Design review of the part built by this model. Coordinates are the model's own, in mm. A direction names the side the tool comes from. Give positions to 0.01 mm unless a question says otherwise; leave off trailing zeros. Write each loop counter-clockwise with the first axis right and the second up, starting at its lowest first coordinate (ties: lowest second). Pieces come first, ordered by that corner, then holes. Notation, with made-up numbers: (84.25, -36.75) -> (110.25, -36.75) arc R13 ccw to (110.25, -17.75) -> close; hole circle Ø4 at (57.25, 76). An arc over 180 degrees is marked (long way). Write each question's results on one line, items separated by ' | '. Start each with the question number.
(1) To check wall thickness, follow probe 1 along Z at (x, y) = (-37.5, 3.25); probe 2 along Z at (x, y) = (-12.5, 16.25); probe 3 along X at (y, z) = (10.25, 7). State the ranges of each line that lie inside material, in increasing order.
(2) Mouldability with a two-part tool opening along Z and no side actions: class faces 4 (the face through (-49.156, 16.181, 49.527)), 5 (the face through (-38.13, 12.98, 38.33)), 6 (the face through (62.5, 5, 0)) as released by +Z, released by -Z, zero draft, split by the parting line, or undercut.
(3) For faces 1 (the face through (-41.15, 5.07, 32.74)), 2 (the face through (53.479, 5.07, 53.945)), 3 (the face through (-7.441, 14.93, 9.274)), list the 3-axis set-ups (+Z, -Z, +X, -X, +Y, -Y) from which the entire face can be reached by the end or side of a thin tool; tool diameter is ignored.
(4) Take a section at A-A (y = 4.5). State the section outline as (x, z) points, plus the area to 3 significant figures.
(5) Take a section at B-B (x = -21.5). State the section outline as (y, z) points.
(6) Take a section at C-C (z = 27.5). State the section outline as (x, y) points.
(7) Clearance check with flat-ended pins moving along their axes: pin 1 (6 mm diameter, centred on x = -41, y = 2.5, fed in from +Z); pin 2 (12 mm diameter, centred on x = 47.5, y = 14.5, fed in from -Z); pin 3 (3 mm diameter, centred on y = 14, z = 6.5, fed in from -X); pin 4 (6 mm diameter, centred on x = -48, z = 23, fed in from -Y). State where each tip first meets the part, or that it passes through.
from build123d import *

# Parameters (mm, degrees)
BASE_PLATE_PROFILE_125X125_W = 125
BASE_PLATE_PROFILE_125X125_H = 125
BASE_PLATE_20MM_DEPTH        = 20
CORNER_FILLETS_R30_R         = 30
EDGE_CHAMFER_10X45_SIZE      = 10
DOWEL_HOLES_12X10_A_D        = 12
DOWEL_HOLES_12X10_A_DEPTH    = 10
DOWEL_HOLES_12X10_A_TIP      = 3.605163714
DOWEL_HOLES_12X10_B_D        = 12
DOWEL_HOLES_12X10_B_DEPTH    = 10
DOWEL_HOLES_12X10_B_TIP      = 3.605163714


with BuildPart() as part:
    # Base Plate Profile 125x125 → Base Plate 20mm (new body)
    with BuildSketch(Plane(origin=(0, 0, 0), x_dir=(1, 0, 0), z_dir=(0, 1, 0))):
        Rectangle(BASE_PLATE_PROFILE_125X125_W, BASE_PLATE_PROFILE_125X125_H)
    extrude(amount=BASE_PLATE_20MM_DEPTH)

    # Corner Fillets R30
    corner_fillets_r30_edges = [part.edges().sort_by_distance(p)[0] for p in [
        (62.5, 10, 62.5),
        (-62.5, 10, 62.5),
        (-62.5, 10, -62.5),
        (62.5, 10, -62.5),
    ]]
    fillet(corner_fillets_r30_edges, radius=CORNER_FILLETS_R30_R)

    # Edge Chamfer 10x45°
    edge_chamfer_10x45_edges = [part.edges().sort_by_distance(p)[0] for p in [
        (-62.5, 20, 0),
        (0, 20, -62.5),
        (62.5, 20, 0),
        (0, 20, 62.5),
        (-53.713203436, 20, 53.713203436),
        (53.713203436, 20, 53.713203436),
        (53.713203436, 20, -53.713203436),
        (-53.713203436, 20, -53.713203436),
    ]]
    chamfer(edge_chamfer_10x45_edges, length=EDGE_CHAMFER_10X45_SIZE)

    # Dowel Holes Ø12x10 A
    with Locations(Plane(origin=(-12.5, 20, -12.5), x_dir=(0, 0, 1), z_dir=(0, 1, 0))):
        with Locations((0, 0), (0, 25), (25, 25), (25, 0)):
            Hole(DOWEL_HOLES_12X10_A_D / 2, depth=DOWEL_HOLES_12X10_A_DEPTH)
            with Locations((0, 0, -(DOWEL_HOLES_12X10_A_DEPTH + DOWEL_HOLES_12X10_A_TIP / 2))):  # 118° drill point
                Cone(0, DOWEL_HOLES_12X10_A_D / 2, DOWEL_HOLES_12X10_A_TIP, mode=Mode.SUBTRACT)

    # Dowel Holes Ø12x10 B
    with Locations(Plane(origin=(-37.5, 0, 37.5), x_dir=(0, 0, -1), z_dir=(0, -1, 0))):
        with Locations((0, 0), (0, 75), (75, 75), (75, 0)):
            Hole(DOWEL_HOLES_12X10_B_D / 2, depth=DOWEL_HOLES_12X10_B_DEPTH)
            with Locations((0, 0, -(DOWEL_HOLES_12X10_B_DEPTH + DOWEL_HOLES_12X10_B_TIP / 2))):  # 118° drill point
                Cone(0, DOWEL_HOLES_12X10_B_D / 2, DOWEL_HOLES_12X10_B_TIP, mode=Mode.SUBTRACT)


solid = part.part
Report:
1) probe 1: -62.08 to -43.5, -31.5 to 31.5, 43.5 to 62.08 | probe 2: -56.25 to -18.5, -6.5 to 6.5, 18.5 to 56.25 | probe 3: -62.25 to -14.9, -10.1 to 10.1, 14.9 to 62.25
2) face 4: released by +Z | face 5: undercut | face 6: zero draft
3) face 1: -Y | face 2: +Z, +X, +Y, -Y | face 3: +Y
4) outline: (-62.5, -32.5) arc R30 ccw to (-32.5, -62.5) -> (32.5, -62.5) arc R30 ccw to (62.5, -32.5) -> (62.5, 32.5) arc R30 ccw to (32.5, 62.5) -> (-32.5, 62.5) arc R30 ccw to (-62.5, 32.5) -> close; hole circle Ø12 at (-37.5, -37.5); hole circle Ø12 at (-37.5, 37.5); hole circle Ø12 at (37.5, -37.5); hole circle Ø12 at (37.5, 37.5) | area: 14,400 mm2
5) outline: (0, -62.5) -> (10, -62.5) -> (20, -52.5) -> (20, 52.5) -> (10, 62.5) -> (0, 62.5) -> close
6) outline: (-62.5, 0) -> (62.5, 0) -> (62.5, 10) -> (52.5, 20) -> (-52.5, 20) -> (-62.5, 10) -> close
7) pin 1: z = 61.99 | pin 2: z = -60.4 | pin 3: x = -60 | pin 4: y = 0
